For this review, take the finished solid that the model builds, in its own axes (mm). A direction names the side the tool comes from. Round coordinates to 2 decimals unless told otherwise and drop trailing zeros. Write each loop counter-clockwise with the first axis right and the second up, starting at its lowest first coordinate (ties: lowest second). Pieces come first, ordered by that corner, then holes. Notation, with made-up numbers: (61, 56.5) - (86, 56.5) arc R15 ccw to (86, 78.5) - close; hole circle Ø11 at (29, -29). An arc over 180 degrees is marked (long way). Answer in a Markdown table with one row per item. Add a question column.
from build123d import *

# Parameters (mm, degrees)
BOSS_EXTRUDE1_START     = 10
SKETCH1_W               = 80
SKETCH1_H               = 80
BOSS_EXTRUDE1_DEPTH     = 50
SKETCH2_W               = 35
SKETCH2_H               = 35
CUT_EXTRUDE1_DEPTH      = 45
SKETCH3_W               = 55
SKETCH3_H               = 55
CUT_EXTRUDE2_DEPTH      = 5
SKETCH4_W               = 15
SKETCH4_H               = 15
CUT_EXTRUDE3_DEPTH      = 156
BOSS_EXTRUDE2_DEPTH     = 10
BOSS_EXTRUDE3_START     = -10
BOSS_EXTRUDE3_DEPTH     = 10
SKETCH9_R               = 4
CUT_EXTRUDE6_DEPTH      = 99
SKETCH13_W              = 35
SKETCH13_H              = 35
CUT_EXTRUDE7_DEPTH      = 200
CUT_EXTRUDE8_DEPTH      = 160.525859973
CUT_EXTRUDE8_DEPTH_BACK = 43
SKETCH14_R              = 2
SKETCH15_W              = 80
SKETCH15_H              = 80
SKETCH15_W_2            = 55
SKETCH15_H_2            = 55
BOSS_EXTRUDE4_DEPTH     = 10


with BuildPart() as part:
    # Sketch1 → Boss-Extrude1 (new body)
    with BuildSketch(Plane.XY.offset(BOSS_EXTRUDE1_START)):
        with Locations((-91.5, -21.5)):
            Rectangle(SKETCH1_W, SKETCH1_H)
    extrude(amount=BOSS_EXTRUDE1_DEPTH)

    # Sketch2 → Cut-Extrude1 (cut)
    with BuildSketch(Plane(origin=(0, 0, 10), x_dir=(-1, 0, 0), z_dir=(0, 0, -1))):
        with Locations((91.5, -21.5)):
            Rectangle(SKETCH2_W, SKETCH2_H)
    extrude(amount=-CUT_EXTRUDE1_DEPTH, mode=Mode.SUBTRACT)

    # Sketch3 → Cut-Extrude2 (cut)
    with BuildSketch(Plane(origin=(0, 0, 10), x_dir=(-1, 0, 0), z_dir=(0, 0, -1))):
        with Locations((91.5, -21.5)):
            Rectangle(SKETCH3_W, SKETCH3_H)
    extrude(amount=-CUT_EXTRUDE2_DEPTH, mode=Mode.SUBTRACT)

    # Sketch4 → Cut-Extrude3 (cut)
    with BuildSketch(Plane(origin=(0, -61.5, 0), x_dir=(-1, 0, 0), z_dir=(0, -1, 0))):
        with Locations((91.5, -27.5)):
            Rectangle(SKETCH4_W, SKETCH4_H)
    extrude(amount=-CUT_EXTRUDE3_DEPTH, mode=Mode.SUBTRACT)

    # Sketch5 → Boss-Extrude2 (add)
    with BuildSketch(Plane.XZ.offset(61.5)):
        with BuildLine():
            Line((-99, 27.5), (-99, 20))
            Line((-99, 20), (-91.499999963, 20))
            ThreePointArc((-91.499999963, 20), (-96.803300846, 22.196699128), (-99, 27.5))
        make_face()
        with BuildLine():
            ThreePointArc((-84, 27.5), (-86.196699128, 22.196699154), (-91.499999963, 20))
            Line((-91.499999963, 20), (-84, 20))
            Line((-84, 20), (-84, 27.5))
        make_face()
        with BuildLine():
            ThreePointArc((-91.5, 35), (-86.196699141, 32.803300859), (-84, 27.5))
            Line((-84, 27.5), (-84, 35))
            Line((-84, 35), (-91.5, 35))
        make_face()
        with BuildLine():
            Line((-99, 35), (-99, 27.5))
            ThreePointArc((-99, 27.5), (-96.803300859, 32.803300859), (-91.5, 35))
            Line((-91.5, 35), (-99, 35))
        make_face()
    extrude(amount=-BOSS_EXTRUDE2_DEPTH)

    # Sketch6 → Boss-Extrude3 (add)
    with BuildSketch(Plane(origin=(0, 18.5, 0), x_dir=(1, 0, 0), z_dir=(0, 1, 0)).offset(BOSS_EXTRUDE3_START)):
        with BuildLine():
            Line((-84, -27.5), (-84, -20))
            Line((-84, -20), (-91.5, -20))
            ThreePointArc((-91.5, -20), (-86.196699141, -22.196699141), (-84, -27.5))
        make_face()
        with BuildLine():
            ThreePointArc((-99, -27.5), (-96.803300859, -22.196699141), (-91.5, -20))
            Line((-91.5, -20), (-99, -20))
            Line((-99, -20), (-99, -27.5))
        make_face()
        with BuildLine():
            ThreePointArc((-91.5, -35), (-96.803300859, -32.803300859), (-99, -27.5))
            Line((-99, -27.5), (-99, -35))
            Line((-99, -35), (-91.5, -35))
        make_face()
        with BuildLine():
            Line((-84, -35), (-84, -27.5))
            ThreePointArc((-84, -27.5), (-86.196699141, -32.803300859), (-91.5, -35))
            Line((-91.5, -35), (-84, -35))
        make_face()
    extrude(amount=BOSS_EXTRUDE3_DEPTH)

    # Sketch9 → Cut-Extrude6 (cut)
    with BuildSketch(Plane.ZY.offset(131.5)):
        with Locations((22, -21.5)):
            Circle(SKETCH9_R)
    extrude(amount=-CUT_EXTRUDE6_DEPTH, mode=Mode.SUBTRACT)

    # Sketch13 → Cut-Extrude7 (cut)
    with BuildSketch(Plane(origin=(0, 0, 55), x_dir=(-1, 0, 0), z_dir=(0, 0, -1))):
        with Locations((91.5, -21.5)):
            Rectangle(SKETCH13_W, SKETCH13_H)
    extrude(amount=-CUT_EXTRUDE7_DEPTH, mode=Mode.SUBTRACT)

    # Sketch14 → Cut-Extrude8 (cut, two sides: drawn at the far end of the back side and taken through both)
    with BuildSketch(Plane(origin=(0, -49, 0), x_dir=(1, 0, 0), z_dir=(0, 1, 0)).offset(-CUT_EXTRUDE8_DEPTH_BACK)):
        with Locations(Location((-91.5, -12.5, 0), (0, 0, 270))):
            Circle(SKETCH14_R)
    extrude(amount=CUT_EXTRUDE8_DEPTH + CUT_EXTRUDE8_DEPTH_BACK, mode=Mode.SUBTRACT)

    # Sketch15 → Boss-Extrude4 (add)
    with BuildSketch(Plane(origin=(0, 0, 10), x_dir=(-1, 0, 0), z_dir=(0, 0, -1))):
        with Locations((91.5, -21.5)):
            Rectangle(SKETCH15_W, SKETCH15_H)
        with Locations((91.5, -21.5)):
            Rectangle(SKETCH15_W_2, SKETCH15_H_2, mode=Mode.SUBTRACT)
    extrude(amount=BOSS_EXTRUDE4_DEPTH)


solid = part.part
Q1. Insertion check: pin 1 Ø2.5 at (x, z) = (-91.5, 12.5) entering from -Y; pin 2 Ø1.5 at (x, y) = (-98.5, 1) entering from -Z. Each pin has a flat end and moves straight along its axis. Give the tip position at first contact, or say it passes through.
Q2. Add section A-A on z = 12.5. State the section outline as (x, y) points.
Q3. Add section D-D on x = -69.5. State the section outline as (y, z) points.
Q4. Add section B-B on y = 12.5. State the section outline as (x, z) points.
Q5. To check wall thickness, follow probe 1 along Y at (x, z) = (-97, 5); probe 2 along X at (y, z) = (-40, 31.5); probe 3 along X at (y, z) = (-9, 31). State the ranges of each line that lie inside material, in increasing order.
Q6. Tool access review of faces 4 (the face through (-109, -22, 37)), 5 (the face through (-91, 2, 35)), 6 (the face through (-64, -22, 8)): name each direction out of +Z, -Z, +X, -X, +Y, -Y from which nothing blocks a thin tool from reaching the whole face with its end or side.
Q7. Draft analysis for pull direction Z (two halves, no side actions). For faces 1 (the face through (-131.5, -22, 30)), 2 (the face through (-73, -21, 15)), 3 (the face through (-86, 8.5, 33)), state which applies: released by +Z, released by -Z, zero draft, split by the parting line, or undercut.
Q8. Add section C-C on x = -107.5. State the section outline as (y, z) points.
Answer sheet:
| question | item | result |
|---|---|---|
| 1 | pin 1 | passes through |
| 1 | pin 2 | stops at z = 15 |
| 2 | outline | (-131.5, -61.5) - (-93.5, -61.5) - (-93.5, -49) - (-119, -49) - (-119, 6) - (-93.5, 6) - (-93.5, 18.5) - (-131.5, 18.5) - close; (-89.5, -61.5) - (-51.5, -61.5) - (-51.5, 18.5) - (-89.5, 18.5) - (-89.5, 6) - (-64, 6) - (-64, -49) - (-89.5, -49) - close |
| 3 | outline | (-61.5, 0) - (-49, 0) - (-49, 15) - (6, 15) - (6, 0) - (18.5, 0) - (18.5, 60) - (-61.5, 60) - close; hole circle Ø8 at (-21.5, 22) |
| 4 | outline | (-131.5, 0) - (-51.5, 0) - (-51.5, 60) - (-131.5, 60) - close; hole circle Ø15 at (-91.5, 27.5); hole circle Ø4 at (-91.5, 12.5) |
| 5 | probe 1 | y = -61.5 to -49, 6 to 18.5 |
| 5 | probe 2 | x = -131.5 to -99, -84 to -51.5 |
| 5 | probe 3 | x = -131.5 to -109, -74 to -51.5 |
| 6 | face 4 | +Z, -Z |
| 6 | face 5 | none |
| 6 | face 6 | -Z |
| 7 | face 1 | zero draft |
| 7 | face 2 | released by -Z |
| 7 | face 3 | undercut |
| 8 | outline | (-61.5, 0) - (-49, 0) - (-49, 15) - (-39, 15) - (-39, 60) - (-61.5, 60) - close; (-4, 15) - (6, 15) - (6, 0) - (18.5, 0) - (18.5, 60) - (-4, 60) - close |
